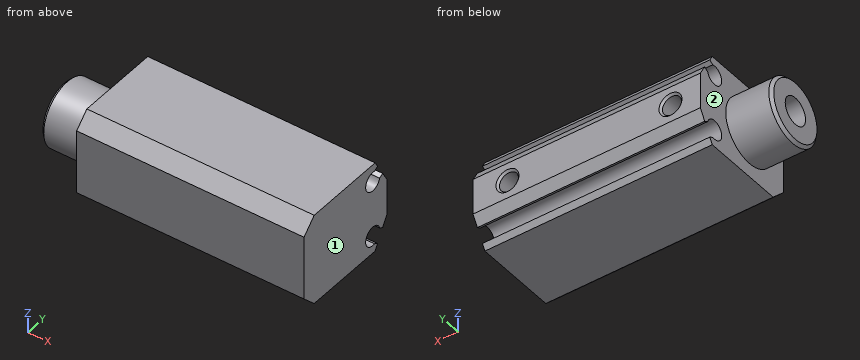
```python
from build123d import *

# Parameters (mm, degrees)
BOSS_EXTRUDE1_DEPTH = 49.5


with BuildPart() as part:
    # Sketch1 → Boss-Extrude1 (new body)
    with BuildSketch(Plane(origin=(0, 0, 0), x_dir=(0, 0, -1), z_dir=(1, 0, 0))):
        with BuildLine():
            Line((-10, -7), (-7, -10))
            Line((-7, -10), (7, -10))
            Line((7, -10), (10, -7))
            Line((10, -7), (10, 10.992597115))
            Line((10, 10.992597115), (8.748941454, 11.714896103))
            Line((8.748941454, 11.714896103), (8.233885029, 10.822792206))
            ThreePointArc((8.233885029, 10.822792206), (5.15, 8.481346652), (5.635808817, 12.322792206))
            Line((5.635808817, 12.322792206), (6.150865242, 13.214896103))
            Line((6.150865242, 13.214896103), (3.925, 14.5))
            Line((3.925, 14.5), (-3.925, 14.5))
            Line((-3.925, 14.5), (-6.150865242, 13.214896103))
            Line((-6.150865242, 13.214896103), (-5.635808817, 12.322792206))
            ThreePointArc((-5.635808817, 12.322792206), (-5.15, 8.481346652), (-8.233885029, 10.822792206))
            Line((-8.233885029, 10.822792206), (-8.748941454, 11.714896103))
            Line((-8.748941454, 11.714896103), (-10, 10.992597115))
            Line((-10, 10.992597115), (-10, -7))
        make_face()
    extrude(amount=BOSS_EXTRUDE1_DEPTH)

    # Sketch2 → Revolve1 (revolve)
    with BuildSketch(Plane.XY, mode=Mode.PRIVATE) as revolve1_sk:
        Polygon((-10, 0), (-10, 6.3865), (-9.3865, 7), (0, 7), (0, 0), align=None)
    revolve(revolve1_sk.sketch.rotate(Axis((0, 0, 0), (-1, 0, 0)), 90), axis=Axis((0, 0, 0), (-1, 0, 0)))

    # Sketch3 → Cut-Revolve1 (revolve, cut)
    with BuildSketch(Plane.XY):
        Polygon((-10, 0), (-10, 3), (11, 3), (11, 8), (38.5, 8), (38.5, 0), align=None)
    revolve(axis=Axis((38.5, 0, 0), (-1, 0, 0)), mode=Mode.SUBTRACT)

    # Sketch4 → Cut-Revolve2 (revolve, cut)
    with BuildSketch(Plane.XY, mode=Mode.PRIVATE) as cut_revolve2_sk:
        Polygon((6.5, 14.5), (9, 14.5), (8.567, 14.067), (8.567, 8.5), (6.5, 7.2580211), align=None)
    revolve(cut_revolve2_sk.sketch.rotate(Axis((6.5, 7.2580211, 0), (0, 1, 0)), 90), axis=Axis((6.5, 7.2580211, 0), (0, 1, 0)), mode=Mode.SUBTRACT)

    # Sketch5 → Cut-Revolve3 (revolve, cut)
    with BuildSketch(Plane.XY, mode=Mode.PRIVATE) as cut_revolve3_sk:
        Polygon((42, 14.5), (44.5, 14.5), (44.067, 14.067), (44.067, 8.5), (42, 7.2580211), align=None)
    revolve(cut_revolve3_sk.sketch.rotate(Axis((42, 7.2580211, 0), (0, 1, 0)), 90), axis=Axis((42, 7.2580211, 0), (0, 1, 0)), mode=Mode.SUBTRACT)


solid = part.part
```
CAD build for the part. Positions are in the model's coordinates, mm. Face numbers are marked on the shaded views. A direction names the side the tool comes from. Round coordinates to 2 decimals unless told otherwise and drop trailing zeros. Write each loop counter-clockwise with the first axis right and the second up, starting at its lowest first coordinate (ties: lowest second). Pieces come first, ordered by that corner, then holes. Notation, with made-up numbers: (28, 19) - (55, 19) arc R9 cw to (55, 27) - close; hole circle Ø9 at (28, -40). An arc over 180 degrees is marked (long way). Return JSON: item names as keys, results as strings. Group by question number.
Item 1: Band-saw the part on B-B on x = 1.5. List the corners of the cut face in (y, z) (3 decimals).
Item 2: Probe probe 1 along X at (y, z) = (-5.5, 3); probe 2 along Y at (x, z) = (4, 0); probe 3 along Z at (x, y) = (22, 10.3). List the from-to ranges inside material, lowest first.
Item 3: Band-saw the part on C-C on z = -5. State how many separate pieces and enclosed holes the cut face has, plus the area to 3 significant figures.
Item 4: Band-saw the part on A-A on x = 31.5. List the corners of the cut face in (y, z) (3 decimals).
Item 5: Flat gauge pins, fed straight in: pin 1 Ø3.5 at (x, z) = (42, 0) entering from +Y; pin 2 Ø2 at (y, z) = (4.5, 7) entering from -X. Where does each tip first touch, or does it go through?
Item 6: 3-axis set-ups, long thin cutter, end or side, ignore diameter. For the marked faces 1 and 2: which of +Z, -Z, +X, -X, +Y, -Y reach the whole face in a straight line?
Resolved:
{
 "1": {"outline": "(-10, -7) - (-7, -10) - (10.993, -10) - (11.715, -8.749) - (10.823, -8.234) arc R2.1 cw (long way) to (12.323, -5.636) - (13.215, -6.151) - (14.5, -3.925) - (14.5, 3.925) - (13.215, 6.151) - (12.323, 5.636) arc R2.1 cw (long way) to (10.823, 8.234) - (11.715, 8.749) - (10.993, 10) - (-7, 10) - (-10, 7) - close; hole circle Ø6 at (0, 0)"},
 "2": {"probe 1": "x = -10 to 11, 38.5 to 49.5", "probe 2": "y = -10 to -3, 3 to 14.5", "probe 3": "z = -10 to -8.3, -4.1 to 4.1, 8.3 to 10"},
 "3": {"separate pieces": "2", "enclosed holes": "1", "area": "765 mm²"},
 "4": {"outline": "(-10, -7) - (-7, -10) - (10.993, -10) - (11.715, -8.749) - (10.823, -8.234) arc R2.1 cw (long way) to (12.323, -5.636) - (13.215, -6.151) - (14.5, -3.925) - (14.5, 3.925) - (13.215, 6.151) - (12.323, 5.636) arc R2.1 cw (long way) to (10.823, 8.234) - (11.715, 8.749) - (10.993, 10) - (-7, 10) - (-10, 7) - close; hole circle Ø16 at (0, 0)"},
 "5": {"pin 1": "stops at y = 8.31", "pin 2": "stops at x = 0"},
 "6": {"face 1": "+Z, -Z, +X, +Y, -Y", "face 2": "-X"}
}
